Read the model definition and answer for the solid it produces. Units are mm, in the model's axes. A direction names the side the tool comes from. Give positions to 0.01 mm unless a question says otherwise; leave off trailing zeros. Order: outer loops, then holes, each group sorted by start corner. A loop starts at its lowest first (then second) coordinate and runs counter-clockwise, first axis right, second up. Notation, with made-up numbers: (-23.5, -34.75) - (14.5, -34.75) arc R5 cw to (14.5, -30.75) - close; hole circle Ø10 at (14.5, 75.25). An arc over 180 degrees is marked (long way). Use a Markdown table: item, result. Add a question column.
1. Flat-ended cylindrical pins translate along their axes: P1, Ø1, axis at y = -172.5, z = 3, coming from the +X side; P2, Ø17.5, axis at x = -348.26, y = -32.72, coming from the +Z side; P3, Ø12, axis at x = -241.53, y = -59.33, coming from the -Z side; P4, Ø1, axis at x = -206, z = 6.5, coming from the +Y side. Find the tip coordinate at first contact, or state that the pin passes through.
2. A cutting plane is placed at C-C on y = -136.5. Determine the outline of the cut face in (x, z).
3. Which of the six approach directions +Z, -Z, +X, -X, +Y, -Y give full straight-line access (tool end or side, diameter ignored) to faces 1 (the conical face through (-128.5, -89.21, 2.89)), 2 (the flat face through (-151.485, 139.285, 3.944))?
4. For a pull along X with two mould halves and no side action, classify faces 3 (the cylindrical face through (371.628, -76.897, 3.944)), 4 (the flat face through (90, 90, 8)), 5 (the flat face through (-204.122, -50.622, 3.944)) as released by +X, released by -X, zero draft, split by the parting line, or undercut.
5. A cutting plane is placed at A-A on z = 4.75. State how many separate pieces and enclosed holes the cut face has, and give its area (3 significant figures).
6. A cutting plane is placed at B-B on x = 0. Determine the outline of the cut face in (y, z), and give its area (3 significant figures).
7. Consider L1, parallel to Y at x = -239.5, z = 2.5; L2, parallel to Y at x = -177.5, z = 6.75; L3, parallel to Y at x = -10, z = 1.5. Determine where each line is inside the solid, lowest interval first.
```python
from build123d import *

# Parameters (mm, degrees)
BOSS_EXTRUDE1_DEPTH                        = 8
HOLE_SIZE_PER_FOR_TYPE_1_HEX_SOCK_2_COUNT  = 2
HOLE_SIZE_PER_FOR_TYPE_1_HEX_SOCK_2_PITCH  = 110
HOLE_SIZE_PER_FOR_TYPE_1_HEX_SOCK_3_COUNT  = 2
HOLE_SIZE_PER_FOR_TYPE_1_HEX_SOCK_3_PITCH  = 220
HOLE_SIZE_PER_FOR_TYPE_1_HEX_SOCK_4_COUNT  = 2
HOLE_SIZE_PER_FOR_TYPE_1_HEX_SOCK_4_PITCH  = 330
HOLE_SIZE_PER_FOR_TYPE_1_HEX_SOCK_5_COUNT  = 2
HOLE_SIZE_PER_FOR_TYPE_1_HEX_SOCK_5_PITCH  = 434.348828609
HOLE_SIZE_PER_FOR_TYPE_1_HEX_SOCK_6_COUNT  = 2
HOLE_SIZE_PER_FOR_TYPE_1_HEX_SOCK_6_PITCH  = 464.296139241
HOLE_SIZE_PER_FOR_TYPE_1_HEX_SOCK_7_COUNT  = 2
HOLE_SIZE_PER_FOR_TYPE_1_HEX_SOCK_7_PITCH  = 403.390629539
HOLE_SIZE_PER_FOR_TYPE_1_HEX_SOCK_8_COUNT  = 2
HOLE_SIZE_PER_FOR_TYPE_1_HEX_SOCK_8_PITCH  = 319.724881734
HOLE_SIZE_PER_FOR_TYPE_1_HEX_SOCK_9_COUNT  = 2
HOLE_SIZE_PER_FOR_TYPE_1_HEX_SOCK_9_PITCH  = 256.756694168
HOLE_SIZE_PER_FOR_TYPE_1_HEX_SOCK_10_COUNT = 2
HOLE_SIZE_PER_FOR_TYPE_1_HEX_SOCK_10_PITCH = 232


with BuildPart() as part:
    # Sketch1 → Boss-Extrude1 (new body)
    with BuildSketch(Plane.XY):
        with BuildLine():
            Line((23.829306717, 95.574129038), (-331.778451057, 184.237101079))
            ThreePointArc((-331.778451057, 184.237101079), (368.227228122, -91.80935938), (-379.43706449, -6.911156997))
            Line((-379.43706449, -6.911156997), (-23.829306717, -95.574129038))
            ThreePointArc((-23.829306717, -95.574129038), (95.574129038, -23.829306717), (23.829306717, 95.574129038))
        make_face()
    extrude(amount=BOSS_EXTRUDE1_DEPTH)

    # Sketch6 → Hole size (per %) for Type 1 hex socket Torx semi-countersunk screw (revolve, cut)
    with BuildSketch(Plane(origin=(-292.134649782, 192.388529796, 8), x_dir=(0, -1, 0), z_dir=(1, 0, 0))):
        Polygon((0, 0), (0, 8), (6.75, 8), (6.75, 5.45), (12.2, 0), align=None)
    hole_size_per_for_type_1_hex_socket_t = revolve(axis=Axis((-292.134649782, 192.388529796, 14.35), (0, 0, -1)), mode=Mode.SUBTRACT)

    # Hole size _per _ for Type 1 hex sock 2: Hole size (per %) for Type 1 hex socket Torx semi-countersunk screw ×2
    with Locations(*[Vector(0.9702957262760132, -0.24192189559960064, 0) * (i * HOLE_SIZE_PER_FOR_TYPE_1_HEX_SOCK_2_PITCH) for i in range(1, HOLE_SIZE_PER_FOR_TYPE_1_HEX_SOCK_2_COUNT)]):
        add(hole_size_per_for_type_1_hex_socket_t, mode=Mode.SUBTRACT)

    # Hole size _per _ for Type 1 hex sock 3: Hole size (per %) for Type 1 hex socket Torx semi-countersunk screw ×2
    with Locations(*[Vector(0.9702957262760132, -0.24192189559960078, 0) * (i * HOLE_SIZE_PER_FOR_TYPE_1_HEX_SOCK_3_PITCH) for i in range(1, HOLE_SIZE_PER_FOR_TYPE_1_HEX_SOCK_3_COUNT)]):
        add(hole_size_per_for_type_1_hex_socket_t, mode=Mode.SUBTRACT)

    # Hole size _per _ for Type 1 hex sock 4: Hole size (per %) for Type 1 hex socket Torx semi-countersunk screw ×2
    with Locations(*[Vector(0.9702957262760132, -0.24192189559960064, 0) * (i * HOLE_SIZE_PER_FOR_TYPE_1_HEX_SOCK_4_PITCH) for i in range(1, HOLE_SIZE_PER_FOR_TYPE_1_HEX_SOCK_4_COUNT)]):
        add(hole_size_per_for_type_1_hex_socket_t, mode=Mode.SUBTRACT)

    # Hole size _per _ for Type 1 hex sock 5: Hole size (per %) for Type 1 hex socket Torx semi-countersunk screw ×2
    with Locations(*[Vector(0.9293014736642066, -0.36932204245825073, 0) * (i * HOLE_SIZE_PER_FOR_TYPE_1_HEX_SOCK_5_PITCH) for i in range(1, HOLE_SIZE_PER_FOR_TYPE_1_HEX_SOCK_5_COUNT)]):
        add(hole_size_per_for_type_1_hex_socket_t, mode=Mode.SUBTRACT)

    # Hole size _per _ for Type 1 hex sock 6: Hole size (per %) for Type 1 hex socket Torx semi-countersunk screw ×2
    with Locations(*[Vector(0.8089192109912862, -0.587919816037217, 0) * (i * HOLE_SIZE_PER_FOR_TYPE_1_HEX_SOCK_6_PITCH) for i in range(1, HOLE_SIZE_PER_FOR_TYPE_1_HEX_SOCK_6_COUNT)]):
        add(hole_size_per_for_type_1_hex_socket_t, mode=Mode.SUBTRACT)

    # Hole size _per _ for Type 1 hex sock 7: Hole size (per %) for Type 1 hex socket Torx semi-countersunk screw ×2
    with Locations(*[Vector(0.6546302530469048, -0.7559492256730906, 0) * (i * HOLE_SIZE_PER_FOR_TYPE_1_HEX_SOCK_7_PITCH) for i in range(1, HOLE_SIZE_PER_FOR_TYPE_1_HEX_SOCK_7_COUNT)]):
        add(hole_size_per_for_type_1_hex_socket_t, mode=Mode.SUBTRACT)

    # Hole size _per _ for Type 1 hex sock 8: Hole size (per %) for Type 1 hex socket Torx semi-countersunk screw ×2
    with Locations(*[Vector(0.49210802471224957, -0.8705341417852651, 0) * (i * HOLE_SIZE_PER_FOR_TYPE_1_HEX_SOCK_8_PITCH) for i in range(1, HOLE_SIZE_PER_FOR_TYPE_1_HEX_SOCK_8_COUNT)]):
        add(hole_size_per_for_type_1_hex_socket_t, mode=Mode.SUBTRACT)

    # Hole size _per _ for Type 1 hex sock 9: Hole size (per %) for Type 1 hex socket Torx semi-countersunk screw ×2
    with Locations(*[Vector(0.19709963269028047, -0.9803834631374382, 0) * (i * HOLE_SIZE_PER_FOR_TYPE_1_HEX_SOCK_9_PITCH) for i in range(1, HOLE_SIZE_PER_FOR_TYPE_1_HEX_SOCK_9_COUNT)]):
        add(hole_size_per_for_type_1_hex_socket_t, mode=Mode.SUBTRACT)

    # Hole size _per _ for Type 1 hex sock 10: Hole size (per %) for Type 1 hex socket Torx semi-countersunk screw ×2
    with Locations(*[Vector(-0.24192189559966096, -0.9702957262759981, 0) * (i * HOLE_SIZE_PER_FOR_TYPE_1_HEX_SOCK_10_PITCH) for i in range(1, HOLE_SIZE_PER_FOR_TYPE_1_HEX_SOCK_10_COUNT)]):
        add(hole_size_per_for_type_1_hex_socket_t, mode=Mode.SUBTRACT)


solid = part.part
```
Output values:
| question | item | result |
|---|---|---|
| 1 | P1 | x = 338.28 |
| 1 | P2 | z = 4.55 |
| 1 | P3 | through |
| 1 | P4 | y = 319.05 |
| 2 | outline | (-354.1, 0) - (354.1, 0) - (354.1, 8) - (-354.1, 8) - close |
| 3 | face 1 | +Z |
| 3 | face 2 | +Z, -Z, -X |
| 4 | face 3 | split by the parting line |
| 4 | face 4 | zero draft |
| 4 | face 5 | undercut |
| 5 | separate pieces | 1 |
| 5 | enclosed holes | 10 |
| 5 | area | 361,000 mm² |
| 6 | outline | (-379.5, 0) - (-98.5, 0) - (-98.5, 8) - (-379.5, 8) - close; (101.52, 0) - (379.5, 0) - (379.5, 8) - (101.52, 8) - close |
| 6 | area | 4,470 mm² |
| 7 | L1 | -294.38 to -65.77, -52.89 to -41.8, 161.23 to 294.38 |
| 7 | L2 | -335.43 to -57.26, 145.77 to 158.2, 173.36 to 335.43 |
| 7 | L3 | -379.37 to -97.99, 104.01 to 379.37 |
